```python
from build123d import *

# Parameters (mm, degrees)
SKETCH_1_4_R       = 52.5
EXTRUDE1_DEPTH     = 30
SKETCH_1_3_R       = 30
EXTRUDE2_DEPTH     = 18
CUT_EXTRUDE1_DEPTH = 87.962635655
CHAMFER1_SIZE      = 1


with BuildPart() as part:
    # Sketch 1_4 → Extrude1 (new body)
    with BuildSketch(Plane.XY):
        with Locations((0, 10)):
            Circle(SKETCH_1_4_R)
    extrude(amount=EXTRUDE1_DEPTH)

    # 草图1<3> → Extrude2 (add)
    with BuildSketch(Plane.XY):
        Circle(SKETCH_1_3_R)
        with BuildLine():
            Line((5, 19.364916731), (5, 23.3))
            Line((5, 23.3), (-5, 23.3))
            Line((-5, 23.3), (-5, 19.364916731))
            ThreePointArc((-5, 19.364916731), (0, -20), (5, 19.364916731))
        make_face(mode=Mode.SUBTRACT)
    extrude(amount=-EXTRUDE2_DEPTH)

    # Sketch 1_4 2 → Cut-Extrude1 (cut, through all)
    with BuildSketch(Plane.XY):
        with BuildLine():
            Line((5, 19.364916731), (5, 23.3))
            Line((5, 23.3), (-5, 23.3))
            Line((-5, 23.3), (-5, 19.364916731))
            ThreePointArc((-5, 19.364916731), (0, -20), (5, 19.364916731))
        make_face()
    extrude(amount=CUT_EXTRUDE1_DEPTH, mode=Mode.SUBTRACT)

    # Chamfer1
    chamfer1_edges = [part.edges().sort_by_distance(p)[0] for p in [
        (-52.5, 10, 0),
        (0, -20, 30),
        (-52.5, 10, 30),
        (-30, 0, -18),
        (0, -20, -18),
    ]]
    chamfer(chamfer1_edges, length=CHAMFER1_SIZE)


solid = part.part
```
Can you work these out from the model? Positions are in its coordinate system, mm. A direction names the side the tool comes from. Give positions to 0.01 mm unless a question says otherwise; leave off trailing zeros. Order: outer loops, then holes, each group sorted by start corner. A loop starts at its lowest first (then second) coordinate and runs counter-clockwise, first axis right, second up. Notation, with made-up numbers: (48, -29.5) - (73, -29.5) arc R13 cw to (73, -5.5) - close; hole circle Ø3 at (-16, 19.5). An arc over 180 degrees is marked (long way). Use a Markdown table: item, result. Add a question column.
Q1. If we section it at B-B on z = 19: Write out the boundary of the cut face in (x, y), plus the area to 3 significant figures.
Q2. If we section it at A-A on x = 0: Write out the boundary of the cut face in (y, z), plus the area to 3 significant figures.
Q3. If we mould it in two halves opening along Y, with no side actions, what happens to faces 4 (the flat face through (0, 23.3, 6)), 5 (the flat face through (-1, 34, 0)), 6 (the cylindrical face through (-6.834, 62.053, 14.804))? For each: released by +Y, released by -Y, zero draft, split by the parting line, or undercut.
Q4. I'm going to push flat-ended pins straight in: pin 1 (12 mm diameter, centred on x = -12.5, y = 4.5, fed in from -Z); pin 2 (6 mm diameter, centred on y = 17, z = -2.5, fed in from -X); pin 3 (4 mm diameter, centred on x = -2.5, y = 37.5, fed in from -Z); pin 4 (2 mm diameter, centred on y = 22, z = -1.5, fed in from +X). Where does each tip first touch, or does it pass through?
Q5. Please list where these lines run through material, in increasing order: line 1 along Y through (x, z) = (0, 19); line 2 along Z through (x, y) = (13.5, 56); line 3 along Y through (x, z) = (0, -4.5).
Q6. On a 3-axis mill with a long thin cutter (end or side, diameter ignored), from which of +Z, -Z, +X, -X, +Y, -Y can I reach the whole of each face in a straight line? I mean faces 1 (the flat face through (11, 22, 30)), 2 (the flat face through (5, 21, 6)), 3 (the cylindrical face through (-29.97, 1.32, -8.38)). Say none if no direction works.
Answers follow:
| question | item | result |
|---|---|---|
| 1 | outline | circle Ø105 at (0, 10); hole (-5, 19.36) arc R20 ccw (long way) to (5, 19.36) - (5, 23.3) - (-5, 23.3) - close |
| 1 | area | 7,370 mm^2 |
| 2 | outline | (-42.5, 1) - (-41.5, 0) - (-30, 0) - (-30, -17) - (-29, -18) - (-21, -18) - (-20, -17) - (-20, 29) - (-21, 30) - (-41.5, 30) - (-42.5, 29) - close; (23.3, -18) - (29, -18) - (30, -17) - (30, 0) - (61.5, 0) - (62.5, 1) - (62.5, 29) - (61.5, 30) - (23.3, 30) - close |
| 2 | area | 2,150 mm^2 |
| 3 | face 4 | undercut |
| 3 | face 5 | zero draft |
| 3 | face 6 | split by the parting line |
| 4 | pin 1 | passes through |
| 4 | pin 2 | stops at x = -51.55 |
| 4 | pin 3 | stops at z = 0 |
| 4 | pin 4 | stops at x = 21.42 |
| 5 | line 1 | y = -42.5 to -20, 23.3 to 62.5 |
| 5 | line 2 | z = 0 to 30 |
| 5 | line 3 | y = -30 to -20, 23.3 to 30 |
| 6 | face 1 | +Z, +X, -X, +Y, -Y |
| 6 | face 2 | +Z, -Z |
| 6 | face 3 | -Z |
